from build123d import *

# Parameters (mm, degrees)
BOSS_EXTRUDE1_DEPTH = 8


with BuildPart() as part:
    # Sketch1 → Boss-Extrude1 (new body)
    with BuildSketch(Plane.XY):
        with BuildLine():
            Line((-1.538253553, -40.507347935), (-15.538253553, -40.507347935))
            ThreePointArc((-15.538253553, -40.507347935), (-17.538253553, -38.507347935), (-15.538253553, -36.507347935))
            Line((-15.538253553, -36.507347935), (-15.538253553, -35.507347935))
            ThreePointArc((-15.538253553, -35.507347935), (-18.538253553, -38.507347935), (-15.538253553, -41.507347935))
            Line((-15.538253553, -41.507347935), (-1.538253553, -41.507347935))
            Line((-1.538253553, -41.507347935), (-1.538253553, -40.507347935))
        make_face()
    extrude(amount=BOSS_EXTRUDE1_DEPTH)


solid = part.part
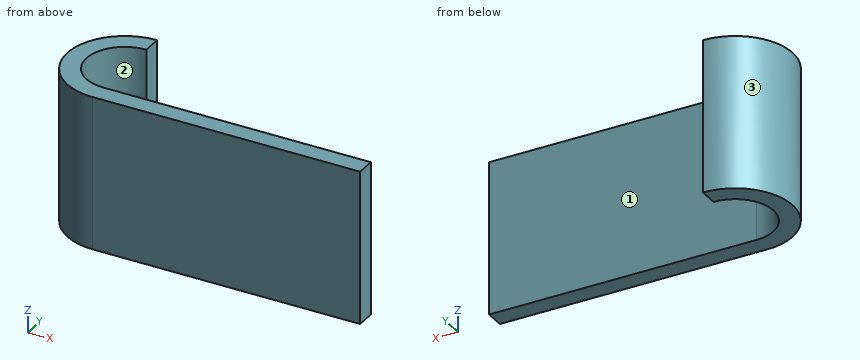
Check sheet for the modelled part. Datum: model origin and axes. Units: mm. Face numbers are marked on the shaded views. Give positions to 0.01 mm unless a question says otherwise; leave off trailing zeros. Write each loop counter-clockwise with the first axis right and the second up, starting at its lowest first coordinate (ties: lowest second). Pieces come first, ordered by that corner, then holes. Notation, with made-up numbers: (53.25, -30.75) -> (92.25, -30.75) arc R16 ccw to (92.25, -19.75) -> close; hole circle Ø6 at (45.5, -13). An arc over 180 degrees is marked (long way). Write item = value, one per line.
Item 1: Scan lines: probe 1 along Y at (x, z) = (-7, 1.5); probe 2 along Y at (x, z) = (-16.5, 2.25); probe 3 along Y at (x, z) = (-16, 3.75). Record each from-to range of solid material in increasing order. Write a range as from..to.
Output:
probe_1 = -41.51..-40.51
probe_2 = -41.35..-40.26, -36.75..-35.67
probe_3 = -41.47..-40.45, -36.56..-35.54
Item 2: Sectioned sample at A-A on x = -6.75. Record the boundary of the cut face in (y, z), and give its area (3 significant figures).
Output:
outline = (-41.51, 0) -> (-40.51, 0) -> (-40.51, 8) -> (-41.51, 8) -> close
area = 8.00 mm^2
Item 3: Sectioned sample at C-C on y = -39.1. Record the boundary of the cut face in (x, z).
Output:
outline = (-18.48, 0) -> (-17.45, 0) -> (-17.45, 8) -> (-18.48, 8) -> close
Item 4: Sectioned sample at B-B on z = 1.75. Record the boundary of the cut face in (x, y).
Output:
outline = (-15.54, -41.51) -> (-1.54, -41.51) -> (-1.54, -40.51) -> (-15.54, -40.51) arc R2 cw to (-15.54, -36.51) -> (-15.54, -35.51) arc R3 ccw to start
Item 5: Gauge pin test, flat ends, axial feed: pin 1 (1 mm diameter, centred on y = -39, z = 1, fed in from +X); pin 2 (1.5 mm diameter, centred on y = -39, z = 5.5, fed in from +X); pin 3 (2 mm diameter, centred on x = -5, z = 1, fed in from +Y). Record the tip position at first contact, or that the pin passes through.
Output:
pin_1 = -17.27
pin_2 = -17.11
pin_3 = -40.51
Item 6: Release check for a two-part mould opening along Y. For the marked faces 1, 2 and 3 record: +Y half, -Y half, draft (parallel to the pull), parting line (faces both ways), or undercut.
Output:
face_1 = +Y half
face_2 = undercut
face_3 = parting line
